Geometry: final body of the model. Coordinates: model frame, mm. Give positions to 0.01 mm unless a question says otherwise; leave off trailing zeros. Order: outer loops, then holes, each group sorted by start corner. A loop starts at its lowest first (then second) coordinate and runs counter-clockwise, first axis right, second up. Notation, with made-up numbers: (-18.5, -3) - (17.5, -3) arc R23 ccw to (17.5, 28) - close; hole circle Ø10 at (-31, -31). An arc over 180 degrees is marked (long way). Use one line per item in the form item = value.
from build123d import *

# Parameters (mm, degrees)
SKETCH1_R              = 12.5
BOSS_EXTRUDE1_DEPTH    = 166
FILLET1_R              = 2
M12_TAPPED_HOLE1_D     = 10.2
M12_TAPPED_HOLE1_DEPTH = 30
M12_TAPPED_HOLE1_TIP   = 3.064389157
M12_TAPPED_HOLE2_D     = 10.2
M12_TAPPED_HOLE2_DEPTH = 30
M12_TAPPED_HOLE2_TIP   = 3.064389157


with BuildPart() as part:
    # Sketch1 → Boss-Extrude1 (new body)
    with BuildSketch(Plane.XY):
        Circle(SKETCH1_R)
    extrude(amount=BOSS_EXTRUDE1_DEPTH)

    # Fillet1
    fillet1_edges = [part.edges().sort_by_distance(p)[0] for p in [
        (-12.5, 0, 0),
        (-12.5, 0, 166),
    ]]
    fillet(fillet1_edges, radius=FILLET1_R)

    # M12 Tapped Hole1
    with Locations(Plane.XY.offset(166)):
        with Locations((0, 0)):
            Hole(M12_TAPPED_HOLE1_D / 2, depth=M12_TAPPED_HOLE1_DEPTH)
            with Locations((0, 0, -(M12_TAPPED_HOLE1_DEPTH + M12_TAPPED_HOLE1_TIP / 2))):  # 118° drill point
                Cone(0, M12_TAPPED_HOLE1_D / 2, M12_TAPPED_HOLE1_TIP, mode=Mode.SUBTRACT)

    # M12 Tapped Hole2
    with Locations(Plane(origin=(0, 0, 0), x_dir=(-1, 0, 0), z_dir=(0, 0, -1))):
        with Locations((0, 0)):
            Hole(M12_TAPPED_HOLE2_D / 2, depth=M12_TAPPED_HOLE2_DEPTH)
            with Locations((0, 0, -(M12_TAPPED_HOLE2_DEPTH + M12_TAPPED_HOLE2_TIP / 2))):  # 118° drill point
                Cone(0, M12_TAPPED_HOLE2_D / 2, M12_TAPPED_HOLE2_TIP, mode=Mode.SUBTRACT)


solid = part.part
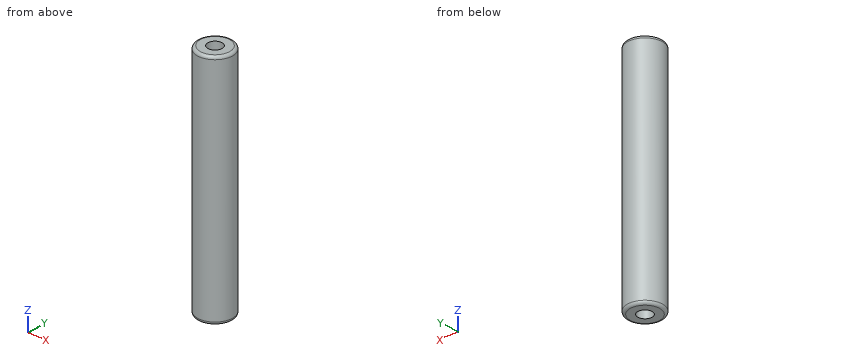
(1) Ray query, line 1 along Y through (x, z) = (0, 143.5); line 2 along X through (y, z) = (2.25, 153); line 3 along X through (y, z) = (0.25, 104.5). Return the intervals inside material, ascending.
Computed values:
line_1 = -12.5 to -5.1, 5.1 to 12.5
line_2 = -12.3 to -4.58, 4.58 to 12.3
line_3 = -12.5 to 12.5
(2) Cut plane A-A on z = 68. Output: boundary loops of the cut face in (x, y).
Computed values:
outline = circle Ø25 at (0, 0)
(3) Contact query for flat-ended pins moving along their axis: pin 1 Ø3 at (y, z) = (1.5, 17) entering from +X; pin 2 Ø1.5 at (y, z) = (4, 116.5) entering from -X; pin 3 Ø8 at (x, y) = (0, 0) entering from +Z; pin 4 Ø5 at (x, z) = (4.5, 149) entering from +Y. Output: stop coordinate, or through.
Computed values:
pin_1 = 12.5
pin_2 = -12.07
pin_3 = 135.34
pin_4 = 12.34
